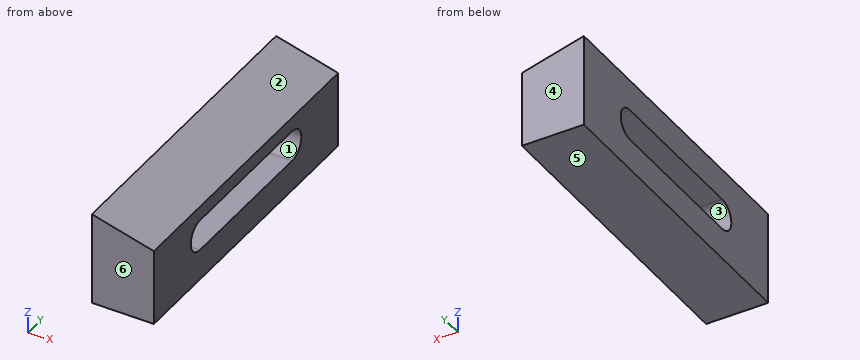
```python
from build123d import *

# Parameters (mm, degrees)
SKETCH1_W           = 60
SKETCH1_H           = 200
BOSS_EXTRUDE1_DEPTH = 20
CUT_EXTRUDE1_DEPTH  = 210.761769634


with BuildPart() as part:
    # Sketch1 → Boss-Extrude1 (new, symmetric)
    with BuildSketch(Plane(origin=(0, 0, 0), x_dir=(0, 0, -1), z_dir=(1, 0, 0))):
        with Locations((30, 100)):
            Rectangle(SKETCH1_W, SKETCH1_H)
        with BuildLine():
            Line((20, 50), (20, 150))
            ThreePointArc((20, 150), (30, 160), (40, 150))
            Line((40, 150), (40, 50))
            ThreePointArc((40, 50), (30, 40), (20, 50))
        make_face(mode=Mode.SUBTRACT)
    extrude(amount=BOSS_EXTRUDE1_DEPTH, both=True)

    # Sketch3 → Cut-Extrude1 (cut, through all)
    with BuildSketch(Plane.XZ):
        Polygon((-20, 0), (20, -10.717967697), (20, 0), align=None)
    extrude(amount=-CUT_EXTRUDE1_DEPTH, mode=Mode.SUBTRACT)


solid = part.part
```
Geometry check sheet. Reference: the model listing, model coordinates, mm. Face numbers are marked on the shaded views. A direction names the side the tool comes from. Round coordinates to 2 decimals unless told otherwise and drop trailing zeros. Loops run counter-clockwise (first coordinate to the right, second up) from the corner with the lowest first, then second, coordinate; pieces in that order, holes last. Notation, with made-up numbers: (55.25, 72.25) - (94.25, 72.25) arc R10 ccw to (94.25, 84.25) - close; hole circle Ø6 at (-8.5, 37.5). An arc over 180 degrees is marked (long way). Use a Markdown table: item, result.
Q1. Material ranges on line 1 (Y direction, x = -18, z = -29.5); line 2 (Z direction, x = -3, y = 79); line 3 (Z direction, x = 1, y = 57), recorded low to high.
Solutions:
| item | result |
|---|---|
| line 1 | y = 0 to 40.01, 159.99 to 200 |
| line 2 | z = -60 to -40, -20 to -4.56 |
| line 3 | z = -60 to -40, -20 to -5.63 |
Q2. Cross-section at C-C on x = 12. Record the cut outline in (y, z).
Solutions:
| item | result |
|---|---|
| outline | (0, -60) - (200, -60) - (200, -8.57) - (0, -8.57) - close; hole (50, -40) - (150, -40) arc R10 ccw to (150, -20) - (50, -20) arc R10 ccw to start |
Q3. Cross-section at D-D on y = 17. Record the cut outline in (x, z).
Solutions:
| item | result |
|---|---|
| outline | (-20, -60) - (20, -60) - (20, -10.72) - (-20, 0) - close |
Q4. Cross-section at B-B on z = -30. Record the cut outline in (x, y).
Solutions:
| item | result |
|---|---|
| outline | (-20, 0) - (20, 0) - (20, 40) - (-20, 40) - close; (-20, 160) - (20, 160) - (20, 200) - (-20, 200) - close |
Q5. Access from +Z, -Z, +X, -X, +Y, -Y to the whole of each face (thin tool, end or side, straight path). Record for the marked faces 1 and 2.
Solutions:
| item | result |
|---|---|
| face 1 | +X, -X |
| face 2 | +Z, +X, +Y, -Y |
Q6. Go/stop test with flat-tipped pins: P1, Ø10, axis at x = -4, y = 159.5, coming from the +Z side; P2, Ø1.5, axis at x = 2.5, y = 163, coming from the +Z side; P3, Ø12, axis at x = 1, y = 122, coming from the +Z side. Record where each tip stops, or that it passes through.
Solutions:
| item | result |
|---|---|
| P1 | stops at z = -2.95 |
| P2 | stops at z = -5.83 |
| P3 | stops at z = -4.02 |
Q7. Draft check along Y on the marked faces 3, 4, 5 and 6. Enter one of: released by +Y, released by -Y, zero draft, split by the parting line, or undercut.
Solutions:
| item | result |
|---|---|
| face 3 | undercut |
| face 4 | released by +Y |
| face 5 | zero draft |
| face 6 | released by -Y |
Q8. Cross-section at A-A on y = 72. Record the cut outline in (x, z), plus the area to 3 significant figures.
Solutions:
| item | result |
|---|---|
| outline | (-20, -60) - (20, -60) - (20, -40) - (-20, -40) - close; (-20, -20) - (20, -20) - (20, -10.72) - (-20, 0) - close |
| area | 1,390 mm2 |
